Source: CAD feature listing. Evaluate the final solid. Frame: model axes, mm. A direction names the side the tool comes from. Give positions to 0.01 mm unless a question says otherwise; leave off trailing zeros. Write each loop counter-clockwise with the first axis right and the second up, starting at its lowest first coordinate (ties: lowest second). Pieces come first, ordered by that corner, then holes. Notation, with made-up numbers: (-29.5, -10) -> (6.5, -10) arc R10 cw to (6.5, 8) -> close; hole circle Ø2 at (89.25, 53.5). An arc over 180 degrees is marked (long way). Write item = value, one per line.
from build123d import *

# Parameters (mm, degrees)
SKETCH1_W                      = 53
SKETCH1_H                      = 11
BOSS_EXTRUDE1_DEPTH            = 6
F_10_0_10_DIAMETER_HOLE1_D     = 10
F_10_0_10_DIAMETER_HOLE1_DEPTH = 14
FILLET1_R                      = 4


with BuildPart() as part:
    # Sketch1 → Revolve1 (revolve)
    with BuildSketch(Plane.XY, mode=Mode.PRIVATE) as revolve1_sk:
        with Locations((26.5, 5.5)):
            Rectangle(SKETCH1_W, SKETCH1_H)
    revolve(revolve1_sk.sketch.rotate(Axis((0, 0, 0), (1, 0, 0)), 270), axis=Axis((0, 0, 0), (1, 0, 0)))

    # Sketch2 → Boss-Extrude1 (add)
    with BuildSketch(Plane.XY.offset(3)):
        Polygon((77, -6), (77, 6), (59, 9), (53, 9), (53, -9), (59, -9), align=None)
    extrude(amount=-BOSS_EXTRUDE1_DEPTH)

    # Ø10.0 (10) Diameter Hole1
    with Locations(Plane(origin=(0, 0, -3), x_dir=(-1, 0, 0), z_dir=(0, 0, -1))):
        with Locations((-69, 0)):
            Hole(F_10_0_10_DIAMETER_HOLE1_D / 2, depth=F_10_0_10_DIAMETER_HOLE1_DEPTH)

    # Sketch5 → CBORE for M13 SHSS1 (revolve, cut)
    with BuildSketch(Plane.ZX):
        Polygon((0, 0), (0, 50), (8, 50), (8, 5), (4, 5), (4, 0), align=None)
    revolve(axis=Axis((-6.35, 0, 0), (1, 0, 0)), mode=Mode.SUBTRACT)

    # Fillet1
    fillet1_edges = [part.edges().sort_by_distance(p)[0] for p in [
        (77, -6, 0),
        (77, 6, 0),
    ]]
    fillet(fillet1_edges, radius=FILLET1_R)


solid = part.part
(1) Section query B-B (z = 0). Return loops of the section in (x, y), plus the area to 3 significant figures.
Values follow:
outline = (0, -11) -> (53, -11) -> (53, -9) -> (59, -9) -> (73.66, -6.56) arc R4 ccw to (77, -2.61) -> (77, 2.61) arc R4 ccw to (73.66, 6.56) -> (59, 9) -> (53, 9) -> (53, 11) -> (0, 11) -> (0, 4) -> (5, 4) -> (5, 8) -> (50, 8) -> (50, -8) -> (5, -8) -> (5, -4) -> (0, -4) -> close; hole circle Ø10 at (69, 0)
area = 701 mm2
(2) Pull-direction query (X, two-part tool) for faces 1 (the face through (56, 9, 0)), 2 (the face through (5, 2, -4)), 3 (the face through (77, 0, 0)); classes: pulls with the +X half, pulls with the -X half, needs draft (parallel to the pull), parting line crosses it, or undercut.
Values follow:
face_1 = needs draft
face_2 = undercut
face_3 = pulls with the +X half
(3) Material intervals for line 1 (Y direction, x = 46, z = 0); line 2 (X direction, y = 0.25, z = 1.75); line 3 (X direction, y = -6.75, z = 3.5), sorted ascending.
Values follow:
line_1 = -11 to -8, 8 to 11
line_2 = 50 to 64.01, 73.99 to 77
line_3 = 0 to 5, 50 to 53
(4) Section query A-A (y = 0). Return loops of the section in (x, z), plus the area to 3 significant figures.
Values follow:
outline = (0, -11) -> (53, -11) -> (53, -3) -> (64, -3) -> (64, 3) -> (53, 3) -> (53, 11) -> (0, 11) -> (0, 4) -> (5, 4) -> (5, 8) -> (50, 8) -> (50, -8) -> (5, -8) -> (5, -4) -> (0, -4) -> close; (74, -3) -> (77, -3) -> (77, 3) -> (74, 3) -> close
area = 490 mm2
(5) Section query C-C (x = 69). Return loops of the section in (y, z).
Values follow:
outline = (-7.33, -3) -> (-5, -3) -> (-5, 3) -> (-7.33, 3) -> close; (5, -3) -> (7.33, -3) -> (7.33, 3) -> (5, 3) -> close
(6) Access query for faces 4 (the face through (27.18, 7.81, -1.73)), 5 (the face through (2.465, 3.905, -0.867)), 6 (the face through (62, 0, -3)). Directions: +Z, -Z, +X, -X, +Y, -Y. A direction counts if a zero-diameter tool reaches every point of the face in a straight line with its end or side. Return the directions, or none.
Values follow:
face_4 = none
face_5 = -X
face_6 = -Z, +X, +Y, -Y
(7) First-contact query: pin 1 (3 mm diameter, centred on x = 59.5, z = -2.5, fed in from +Y); pin 2 (1.8 mm diameter, centred on x = 55.5, z = 1, fed in from -Y); pin 3 (3 mm diameter, centred on x = 27, y = -3, fed in from -Z). Flat tips, straight axial feed; report the tip coordinate or a pass-through.
Values follow:
pin_1 = 9
pin_2 = -9
pin_3 = -10.9
(8) Section query D-D (x = 30.5). Return loops of the section in (y, z), plus the area to 3 significant figures.
Values follow:
outline = circle Ø22 at (0, 0); hole circle Ø16 at (0, 0)
area = 179 mm2
